Here's how the part is built. I have some questions about the finished solid (model axes, mm). A direction names the side the tool comes from. Round coordinates to 2 decimals unless told otherwise and drop trailing zeros. Order: outer loops, then holes, each group sorted by start corner. A loop starts at its lowest first (then second) coordinate and runs counter-clockwise, first axis right, second up. Notation, with made-up numbers: M 39.5,30.25 L 79.5,30.25 A15 cw 79.5,41.25 Z; hole C 61.25,65 d8. An arc over 180 degrees is marked long. Write each question's results on one line, items separated by ' | '. Start each with the question number.
```python
from build123d import *

# Parameters (mm, degrees)
SKETCH1_W           = 30
SKETCH1_H           = 180
BOSS_EXTRUDE1_DEPTH = 2
FILLET1_R           = 10
CUT_EXTRUDE1_DEPTH  = 92.263355187
SKETCH3_R           = 2.75
CUT_EXTRUDE2_DEPTH  = 92.263355187


with BuildPart() as part:
    # Sketch1 → Boss-Extrude1 (new body)
    with BuildSketch(Plane.XY):
        Rectangle(SKETCH1_W, SKETCH1_H)
    extrude(amount=BOSS_EXTRUDE1_DEPTH)

    # Fillet1
    fillet1_edges = [part.edges().sort_by_distance(p)[0] for p in [
        (-15, 90, 1),
        (15, 90, 1),
        (15, -90, 1),
        (-15, -90, 1),
    ]]
    fillet(fillet1_edges, radius=FILLET1_R)

    # Sketch2 → Cut-Extrude1 (cut, through all)
    with BuildSketch(Plane.XY.offset(2)):
        with BuildLine():
            Line((3.5, 80), (3.5, 50))
            ThreePointArc((3.5, 50), (0, 46.5), (-3.5, 50))
            Line((-3.5, 50), (-3.5, 80))
            ThreePointArc((-3.5, 80), (0, 83.5), (3.5, 80))
        make_face()
    cut_extrude1 = extrude(amount=-CUT_EXTRUDE1_DEPTH, mode=Mode.SUBTRACT)

    # Mirror1: Cut-Extrude1 across plane
    add(cut_extrude1.mirror(Plane.ZX), mode=Mode.SUBTRACT)

    # Sketch3 → Cut-Extrude2 (cut, through all)
    with BuildSketch(Plane.XY.offset(2)):
        with Locations((0, -35.5)):
            Circle(SKETCH3_R)
        with Locations((0, 35.5)):
            Circle(SKETCH3_R)
    extrude(amount=-CUT_EXTRUDE2_DEPTH, mode=Mode.SUBTRACT)


solid = part.part
```
(1) Please list where these lines run through material, in increasing order: line 1 (Y direction, x = 0, z = 1.05); line 2 (X direction, y = -77, z = 0.55); line 3 (Y direction, x = 8.5, z = 1.65).
(2) If we mould it in two halves opening along Y, with no side actions, what happens to faces 3 (the cylindrical face through (-0.358, -32.773, 1.014)), 4 (the flat face through (0, 1, 2)), 5 (the cylindrical face through (-12.15, -86.99, 1.01))? For each: pulls with the +Y half, pulls with the -Y half, needs draft (parallel to the pull), parting line crosses it, or undercut.
(3) I want a section at A-A on y = -35.5. Write out the boundary of the cut face in (x, z).
(4) I want a section at B-B on x = 0. Write out the boundary of the cut face in (y, z), and give its area (3 significant figures).
(5) I want a section at C-C on z = 0.75. Write out the boundary of the cut face in (x, y).
(6) I'm going to push a flat-ended pin straight in: pin 1 Ø7 at (x, y) = (0, -35.5) entering from +Z. Where does the tip first touch, or does it pass through?
(7) I want a section at D-D on y = 67. Write out the boundary of the cut face in (x, z).
(8) On a 3-axis mill with a long thin cutter (end or side, diameter ignored), from which of +Z, -Z, +X, -X, +Y, -Y can I reach the whole of each face in a straight line? I mean faces 1 (the cylindrical face through (-12.15, 86.99, 1.01)), 2 (the cylindrical face through (0.1, -46.5, 1)). Say none if no direction works.
Solutions:
1) line 1: -90 to -83.5, -46.5 to -38.25, -32.75 to 32.75, 38.25 to 46.5, 83.5 to 90 | line 2: -15 to -3.5, 3.5 to 15 | line 3: -89.37 to 89.37
2) face 3: undercut | face 4: needs draft | face 5: pulls with the -Y half
3) outline: M -15,0 L -2.75,0 L -2.75,2 L -15,2 Z; M 2.75,0 L 15,0 L 15,2 L 2.75,2 Z
4) outline: M -90,0 L -83.5,0 L -83.5,2 L -90,2 Z; M -46.5,0 L -38.25,0 L -38.25,2 L -46.5,2 Z; M -32.75,0 L 32.75,0 L 32.75,2 L -32.75,2 Z; M 38.25,0 L 46.5,0 L 46.5,2 L 38.25,2 Z; M 83.5,0 L 90,0 L 90,2 L 83.5,2 Z | area: 190 mm^2
5) outline: M -15,-80 A10 ccw -5,-90 L 5,-90 A10 ccw 15,-80 L 15,80 A10 ccw 5,90 L -5,90 A10 ccw -15,80 Z; hole M -3.5,-80 A3.5 ccw 3.5,-80 L 3.5,-50 A3.5 ccw -3.5,-50 Z; hole M -3.5,50 A3.5 ccw 3.5,50 L 3.5,80 A3.5 ccw -3.5,80 Z; hole C 0,-35.5 d5.5; hole C 0,35.5 d5.5
6) pin 1: z = 2
7) outline: M -15,0 L -3.5,0 L -3.5,2 L -15,2 Z; M 3.5,0 L 15,0 L 15,2 L 3.5,2 Z
8) face 1: +Z, -Z, -X, +Y | face 2: +Z, -Z
